Geometry check sheet. Reference: drawing and pictorial views, mm from the part's lowest x, y, z. Coordinates: 2 decimals unless noted, no trailing zeros. Write each loop counter-clockwise with the first axis right and the second up, starting at its lowest first coordinate (ties: lowest second). Pieces come first, ordered by that corner, then holes. Notation, with made-up numbers: (60.25, -30) -> (99.25, -30) arc R17 cw to (99.25, -13) -> close; hole circle Ø5 at (-27.5, -3). An arc over 180 degrees is marked (long way). Use a Markdown table: item, result.
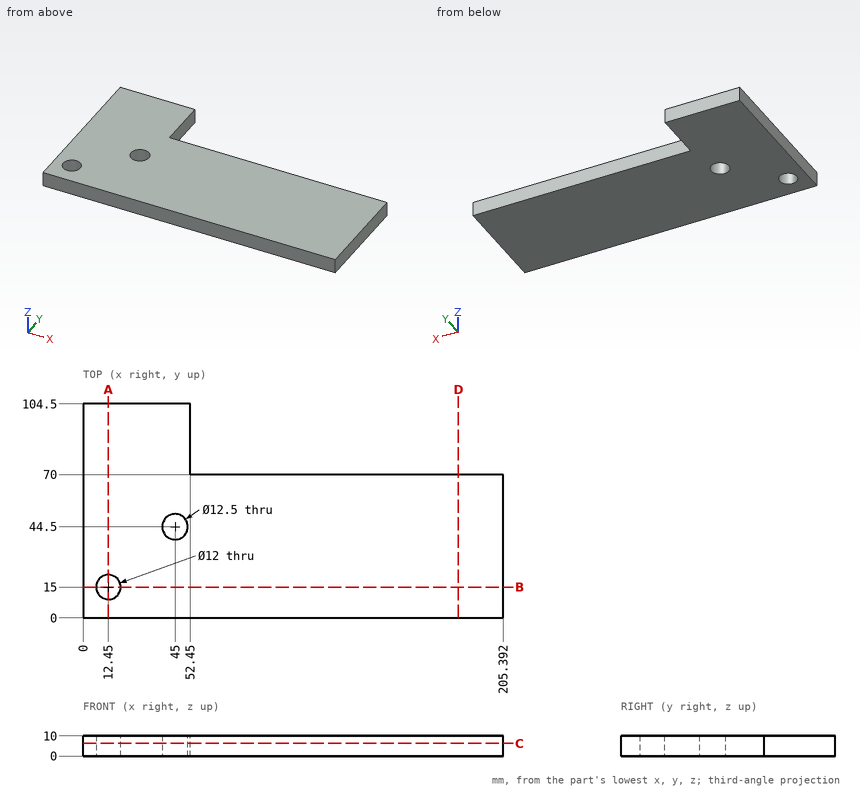
Item 1: Section check A-A on x = 12.45. Record the boundary of the cut face in (y, z), then the cut area to 3 significant figures.
Answer block:
| item | result |
|---|---|
| outline | (0, 0) -> (9, 0) -> (9, 10) -> (0, 10) -> close; (21, 0) -> (104.5, 0) -> (104.5, 10) -> (21, 10) -> close |
| area | 925 mm^2 |
Item 2: Section check B-B on y = 15. Record the boundary of the cut face in (x, z).
Answer block:
| item | result |
|---|---|
| outline | (0, 0) -> (6.45, 0) -> (6.45, 10) -> (0, 10) -> close; (18.45, 0) -> (205.39, 0) -> (205.39, 10) -> (18.45, 10) -> close |
Item 3: Thickness scan on L1, parallel to Y at x = 45, z = 6.75; L2, parallel to Y at x = 12.45, z = 5.5; L3, parallel to X at y = 93, z = 3. Record the ranges inside material, lowest first. Write a range as [from, to].
Answer block:
| item | result |
|---|---|
| L1 | y = [0, 38.25], [50.75, 104.5] |
| L2 | y = [0, 9], [21, 104.5] |
| L3 | x = [0, 52.45] |
Item 4: Section check D-D on x = 183.5. Record the boundary of the cut face in (y, z).
Answer block:
| item | result |
|---|---|
| outline | (0, 0) -> (70, 0) -> (70, 10) -> (0, 10) -> close |
Item 5: Section check C-C on z = 6.25. Record the boundary of the cut face in (x, y).
Answer block:
| item | result |
|---|---|
| outline | (0, 0) -> (205.39, 0) -> (205.39, 70) -> (52.45, 70) -> (52.45, 104.5) -> (0, 104.5) -> close; hole circle Ø12 at (12.45, 15); hole circle Ø12.5 at (45, 44.5) |
Item 6: Depth check by flat-ended pin: P1, Ø5, axis at y = 91.5, z = 5, coming from the +X side; P2, Ø1, axis at x = 60, z = 8.5, coming from the +Y side. Enter the tip coordinate at first touch or a pass-through.
Answer block:
| item | result |
|---|---|
| P1 | stops at x = 52.45 |
| P2 | stops at y = 70 |
